Input: part model. Units: mm. Frame: model coordinates. Face numbers are marked on the shaded views. Give positions to 0.01 mm unless a question says otherwise; leave off trailing zeros. Loops run counter-clockwise (first coordinate to the right, second up) from the corner with the lowest first, then second, coordinate; pieces in that order, holes last. Notation, with made-up numbers: (83.5, 84) - (111.5, 84) arc R21 cw to (111.5, 110) - close; hole circle Ø8 at (-19, -28.5). An arc over 180 degrees is marked (long way). Answer as a JSON object with one key per item and string values. Group by question number.
(1) Section query A-A (x = 72.5). Return loops of the section in (y, z).
(2) Pin query (flat end, axial travel): P1, Ø3, axis at x = 24.5, z = 12, coming from the -Y side. Return the tip coordinate at first contact, or that it passes through.
(3) Mould query, pull axis Y, two halves, no side actions, for the marked faces 1 and 2. Classes: +Y half, -Y half, draft (parallel to the pull), parting line (faces both ways), or undercut.
(4) Section query C-C (z = 13.25). Return loops of the section in (x, y), plus the area to 3 significant figures.
(5) Material intervals for L1, parallel to Y at x = 72.5, z = 13.3; L2, parallel to Z at x = 135.5, y = 126.5; L3, parallel to Y at x = 83, z = 13, sorted ascending.
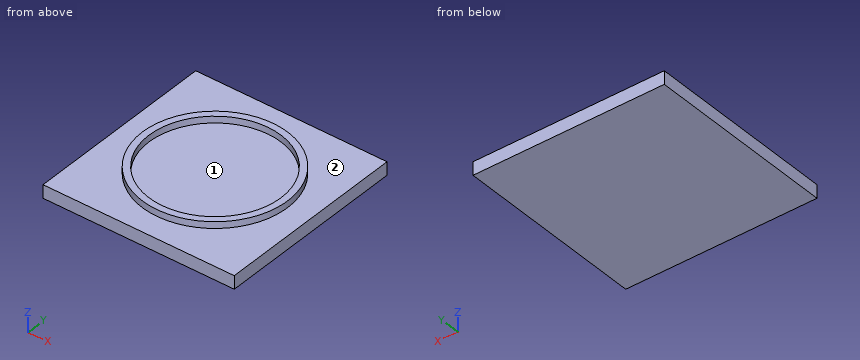
```python
from build123d import *

# Parameters (mm, degrees)
SKETCH1_W           = 145
SKETCH1_H           = 145
BOSS_EXTRUDE1_DEPTH = 10
SKETCH2_R           = 55
SKETCH2_R_2         = 50
BOSS_EXTRUDE2_DEPTH = 5


with BuildPart() as part:
    # Sketch1 → Boss-Extrude1 (new body)
    with BuildSketch(Plane.XY):
        with Locations((72.5, 72.5)):
            Rectangle(SKETCH1_W, SKETCH1_H)
    extrude(amount=BOSS_EXTRUDE1_DEPTH)

    # Sketch2 → Boss-Extrude2 (add)
    with BuildSketch(Plane.XY.offset(10)):
        with Locations(Location((72.5, 72.5, 0), (0, 0, 180))):
            Circle(SKETCH2_R)
        with Locations((72.5, 72.5)):
            Circle(SKETCH2_R_2, mode=Mode.SUBTRACT)
    extrude(amount=BOSS_EXTRUDE2_DEPTH)


solid = part.part
```
Recorded:
{
 "1": {"outline": "(0, 0) - (145, 0) - (145, 10) - (127.5, 10) - (127.5, 15) - (122.5, 15) - (122.5, 10) - (22.5, 10) - (22.5, 15) - (17.5, 15) - (17.5, 10) - (0, 10) - close"},
 "2": {"P1": "stops at y = 43.13"},
 "3": {"face 1": "undercut", "face 2": "draft"},
 "4": {"outline": "circle Ø110 at (72.5, 72.5); hole circle Ø100 at (72.5, 72.5)", "area": "1,650 mm^2"},
 "5": {"L1": "y = 17.5 to 22.5, 122.5 to 127.5", "L2": "z = 0 to 10", "L3": "y = 18.51 to 23.61, 121.39 to 126.49"}
}
